from build123d import *

# Parameters (mm, degrees)
SKETCH1_R             = 35
BOSS_EXTRUDE1_DEPTH   = 10
CHAMFER1_SIZE         = 1
SKETCH2_R             = 1
CUT_EXTRUDE1_DEPTH    = 30
SKETCH3_R             = 4
CUT_EXTRUDE2_DEPTH    = 29
SKETCH4_W             = 8
SKETCH4_H             = 8
CUT_EXTRUDE3_DEPTH    = 51.497524692
FILLET1_R             = 1
SKETCH5_R             = 0.5
CUT_EXTRUDE4_DEPTH    = 54.347914673
SKETCH7_R             = 3
CUT_EXTRUDE5_DEPTH    = 62.040969986
M3_TAPPED_HOLE1_D     = 2.5
M3_TAPPED_HOLE1_DEPTH = 12
M3_TAPPED_HOLE1_TIP   = 0.751075774
CHAMFER2_SIZE         = 0.5


with BuildPart() as part:
    # Sketch1 → Boss-Extrude1 (new body)
    with BuildSketch(Plane.XY):
        Circle(SKETCH1_R)
    extrude(amount=BOSS_EXTRUDE1_DEPTH)

    # Chamfer1
    chamfer1_edges = [part.edges().sort_by_distance(p)[0] for p in [
        (-35, 0, 0),
        (-35, 0, 10),
    ]]
    chamfer(chamfer1_edges, length=CHAMFER1_SIZE)

    # Sketch2 → Cut-Extrude1 (cut)
    with BuildSketch(Plane.XY.offset(10)):
        Circle(SKETCH2_R)
    extrude(amount=-CUT_EXTRUDE1_DEPTH, mode=Mode.SUBTRACT)

    # Sketch3 → Cut-Extrude2 (cut)
    with BuildSketch(Plane.XY.offset(10)):
        with Locations((27.5, 0)):
            Circle(SKETCH3_R)
    extrude(amount=-CUT_EXTRUDE2_DEPTH, mode=Mode.SUBTRACT)

    # Sketch4 → Cut-Extrude3 (cut, through all)
    with BuildSketch(Plane.XY.offset(10)):
        Rectangle(SKETCH4_W, SKETCH4_H)
    extrude(amount=-CUT_EXTRUDE3_DEPTH, mode=Mode.SUBTRACT)

    # Fillet1
    fillet1_edges = [part.edges().sort_by_distance(p)[0] for p in [
        (4, 4, 5),
        (4, -4, 5),
        (-4, -4, 5),
        (-4, 4, 5),
    ]]
    fillet(fillet1_edges, radius=FILLET1_R)

    # Sketch5 → Cut-Extrude4 (cut, through all)
    with BuildSketch(Plane.XZ.offset(-4)):
        with Locations(Location((0, 5, 0), (0, 0, 270))):
            Circle(SKETCH5_R)
    extrude(amount=-CUT_EXTRUDE4_DEPTH, mode=Mode.SUBTRACT)

    # Sketch7 → Cut-Extrude5 (cut, through all)
    with BuildSketch(Plane(origin=(0, 14, 0), x_dir=(1, 0, 0), z_dir=(0, 1, 0))):
        with Locations(Location((0, -5, 0), (0, 0, 90))):
            Circle(SKETCH7_R)
    extrude(amount=CUT_EXTRUDE5_DEPTH, mode=Mode.SUBTRACT)

    # M3 Tapped Hole1
    with Locations(Plane(origin=(0, 14, 5), x_dir=(0, 0, 1), z_dir=(0, 1, 0))):
        with Locations((0, 0)):
            Hole(M3_TAPPED_HOLE1_D / 2, depth=M3_TAPPED_HOLE1_DEPTH)
            with Locations((0, 0, -(M3_TAPPED_HOLE1_DEPTH + M3_TAPPED_HOLE1_TIP / 2))):  # 118° drill point
                Cone(0, M3_TAPPED_HOLE1_D / 2, M3_TAPPED_HOLE1_TIP, mode=Mode.SUBTRACT)

    # Chamfer2
    chamfer2_edges = [part.edges().sort_by_distance(p)[0] for p in [
        (0, -4, 10),
        (0, -4, 0),
        (-4, 0, 10),
        (-4, 0, 0),
        (4, 0, 10),
        (4, 0, 0),
        (0, 4, 10),
        (0, 4, 0),
        (-3.707106781, -3.707106781, 10),
        (-3.707106781, -3.707106781, 0),
        (3.707106781, -3.707106781, 10),
        (3.707106781, -3.707106781, 0),
        (3.707106781, 3.707106781, 10),
        (3.707106781, 3.707106781, 0),
        (-3.707106781, 3.707106781, 10),
        (-3.707106781, 3.707106781, 0),
    ]]
    chamfer(chamfer2_edges, length=CHAMFER2_SIZE)


solid = part.part
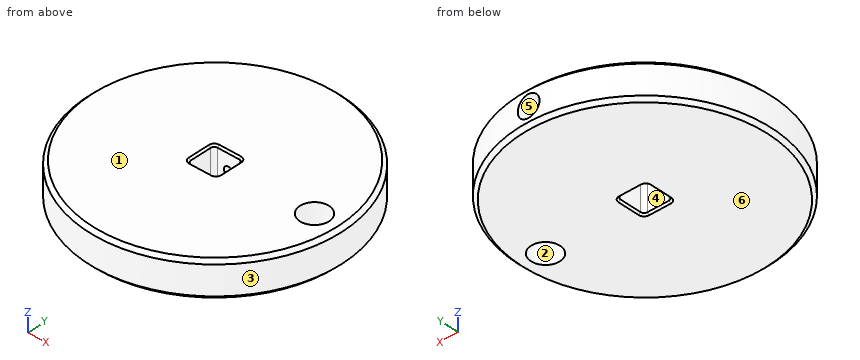
Geometry check sheet. Reference: the model listing, model coordinates, mm. Face numbers are marked on the shaded views. A direction names the side the tool comes from. Round coordinates to 2 decimals unless told otherwise and drop trailing zeros. Order: outer loops, then holes, each group sorted by start corner. A loop starts at its lowest first (then second) coordinate and runs counter-clockwise, first axis right, second up. Notation, with made-up numbers: M -36,29.5 L 4,29.5 A24 cw 4,47.5 Z; hole C -15.5,6.25 d5. An arc over 180 degrees is marked long. Answer in a Markdown table with one row per item.
(1) Scan lines: probe 1 along X at (y, z) = (10, 5.5); probe 2 along X at (y, z) = (-1, 2.25); probe 3 along Y at (x, z) = (27.5, 2.75). Record each from-to range of solid material in increasing order. Write a range as from..to.
Responses:
| item | result |
|---|---|
| probe 1 | x = -33.54..-1.15, 1.15..33.54 |
| probe 2 | x = -34.99..-4, 4..23.63, 31.37..34.99 |
| probe 3 | y = -21.65..-4, 4..21.65 |
(2) Tool access check on the marked faces 4, 5 and 6. Record the directions out of +Z, -Z, +X, -X, +Y, -Y that give a thin tool (end or side, any length) a straight path to the whole face; none if there is none.
Responses:
| item | result |
|---|---|
| face 4 | +Z, -Z |
| face 5 | +Y |
| face 6 | -Z, +X, -X, +Y, -Y |
(3) Sectioned sample at B-B, the plane z = 5. Record the cut outline in (x, y), and give its area (3 significant figures).
Responses:
| item | result |
|---|---|
| outline | M -4,-3 L -4,3 A1 cw -3,4 L -1.25,4 L -1.25,14 L -3,14 L -3,34.87 A35 ccw long 3,34.87 L 3,14 L 1.25,14 L 1.25,4 L 3,4 A1 cw 4,3 L 4,-3 A1 cw 3,-4 L -3,-4 A1 cw Z; hole C 27.5,0 d8 |
| area | 3,580 mm² |
(4) Go/stop test with flat-tipped pins: P1, Ø7, axis at x = 27.5, y = 0, coming from the -Z side; P2, Ø4, axis at y = -13.5, z = 9, coming from the -X side; P3, Ø6, axis at x = -24.5, z = 1, coming from the -Y side; P4, Ø1.8, axis at x = 0, z = 5, coming from the +Y side. Record where each tip stops, or that it passes through.
Responses:
| item | result |
|---|---|
| P1 | passes through |
| P2 | stops at x = -33.06 |
| P3 | stops at y = -27.62 |
| P4 | stops at y = -4 |
(5) Draft check along Y on the marked faces 1, 2 and 3. Enter one of: released by +Y, released by -Y, zero draft, split by the parting line, or undercut.
Responses:
| item | result |
|---|---|
| face 1 | zero draft |
| face 2 | undercut |
| face 3 | split by the parting line |
(6) Sectioned sample at A-A, the plane x = 0. Record the cut outline in (y, z).
Responses:
| item | result |
|---|---|
| outline | M -35,1 L -34,0 L -4.5,0 L -4,0.5 L -4,9.5 L -4.5,10 L -34,10 L -35,9 Z; M 4,0.5 L 4.5,0 L 34,0 L 35,1 L 35,2 L 14,2 L 14,3.75 L 4,3.75 Z; M 4,6.25 L 14,6.25 L 14,8 L 35,8 L 35,9 L 34,10 L 4.5,10 L 4,9.5 Z |
